Input: part model. Units: mm. Frame: model coordinates. A direction names the side the tool comes from. Give positions to 0.01 mm unless a question says otherwise; leave off trailing zeros. Loops run counter-clockwise (first coordinate to the right, second up) from the corner with the lowest first, then second, coordinate; pieces in that order, holes last. Notation, with made-up numbers: (86, 33.25) -> (140, 33.25) arc R33 ccw to (140, 68.25) -> close; hole circle Ø11 at (-31, -26.5). An arc over 180 degrees is marked (long way). Answer in a Markdown table with one row per item. Add a question column.
```python
from build123d import *

# Parameters (mm, degrees)
GROOVE_PROFILE_SKETCH_3X3_W = 3
GROOVE_PROFILE_SKETCH_3X3_H = 4.04600801


with BuildPart() as part:
    # Bushing Profile Sketch → Bushing Body Revolve (revolve)
    with BuildSketch(Plane.XY, mode=Mode.PRIVATE) as bushing_body_revolve_sk:
        Polygon((-9.597352736, 8), (31.902647264, 8), (31.902647264, 16), (28.493054394, 16), (28.493054394, 14), (25.843857713, 14), (25.843857713, 16), (8.402647264, 16), (2.402647264, 13), (-8.597352736, 13), (-9.597352736, 12), align=None)
    revolve(bushing_body_revolve_sk.sketch.rotate(Axis((-43.791817978, 0, 0), (1, 0, 0)), 180), axis=Axis((-43.791817978, 0, 0), (1, 0, 0)))

    # Groove Profile Sketch 3x3 → Groove Cut 3x3 (revolve, cut)
    with BuildSketch(Plane.XY, mode=Mode.PRIVATE) as groove_cut_3x3_sk:
        with Locations((-4.097352736, 13.5210982)):
            Rectangle(GROOVE_PROFILE_SKETCH_3X3_W, GROOVE_PROFILE_SKETCH_3X3_H)
    revolve(groove_cut_3x3_sk.sketch.rotate(Axis((-18.397733025, 0, 0), (1, 0, 0)), 180), axis=Axis((-18.397733025, 0, 0), (1, 0, 0)), mode=Mode.SUBTRACT)


solid = part.part
```
1) Material intervals for line 1 along Z through (x, y) = (14, 0); line 2 along Y through (x, z) = (16, -1); line 3 along X through (y, z) = (-12, 0.5), sorted ascending.
2) Pin query (flat end, axial travel): pin 1 (2 mm diameter, centred on x = -3.5, z = -3.5, fed in from +Y); pin 2 (13 mm diameter, centred on y = 0, z = 0, fed in from -X); pin 3 (4 mm diameter, centred on x = 6.5, y = -2, fed in from +Z); pin 4 (2 mm diameter, centred on y = 12.5, z = -7.5, fed in from -X). Return the tip coordinate at first contact, or that it passes through.
3) Pull-direction query (X, two-part tool) for faces 1 (the face through (25.844, -0.07, 14.15)), 2 (the face through (2.694, -12.539, -3.949)), 3 (the face through (-0.132, 10.316, 7.91)), 4 (the face through (-5.597, 5, 11)); classes: +X half, -X half, draft (parallel to the pull), parting line (faces both ways), or undercut.
4) Reachability of faces 5 (the face through (31.903, -3.8, -7.3)), 6 (the face through (-7.118, 10.316, 7.91)), 7 (the face through (-4.076, -10.621, 4.404)) from +Z, -Z, +X, -X, +Y, -Y: full face, straight path, thin tool, end or side. Return the list, or none.
5) Section C-C on x = 5. Output: boundary loops of the cut face in (y, z).
Working result:
| question | item | result |
|---|---|---|
| 1 | line 1 | z = -16 to -8, 8 to 16 |
| 1 | line 2 | y = -15.97 to -7.94, 7.94 to 15.97 |
| 1 | line 3 | x = -9.59 to -5.6, -2.6 to 31.9 |
| 2 | pin 1 | stops at y = 12.63 |
| 2 | pin 2 | passes through |
| 2 | pin 3 | stops at z = 15.94 |
| 2 | pin 4 | stops at x = 3.56 |
| 3 | face 1 | undercut |
| 3 | face 2 | -X half |
| 3 | face 3 | draft |
| 3 | face 4 | undercut |
| 4 | face 5 | +Z, -Z, +X, +Y, -Y |
| 4 | face 6 | -X |
| 4 | face 7 | none |
| 5 | outline | circle Ø28.6 at (0, 0); hole circle Ø16 at (0, 0) |
